Source: three-view drawing plus pictorial views. Frame: mm from the lowest corner of the part. A direction names the side the tool comes from. Give positions to 0.01 mm unless a question says otherwise; leave off trailing zeros. Loops run counter-clockwise (first coordinate to the right, second up) from the corner with the lowest first, then second, coordinate; pieces in that order, holes last.
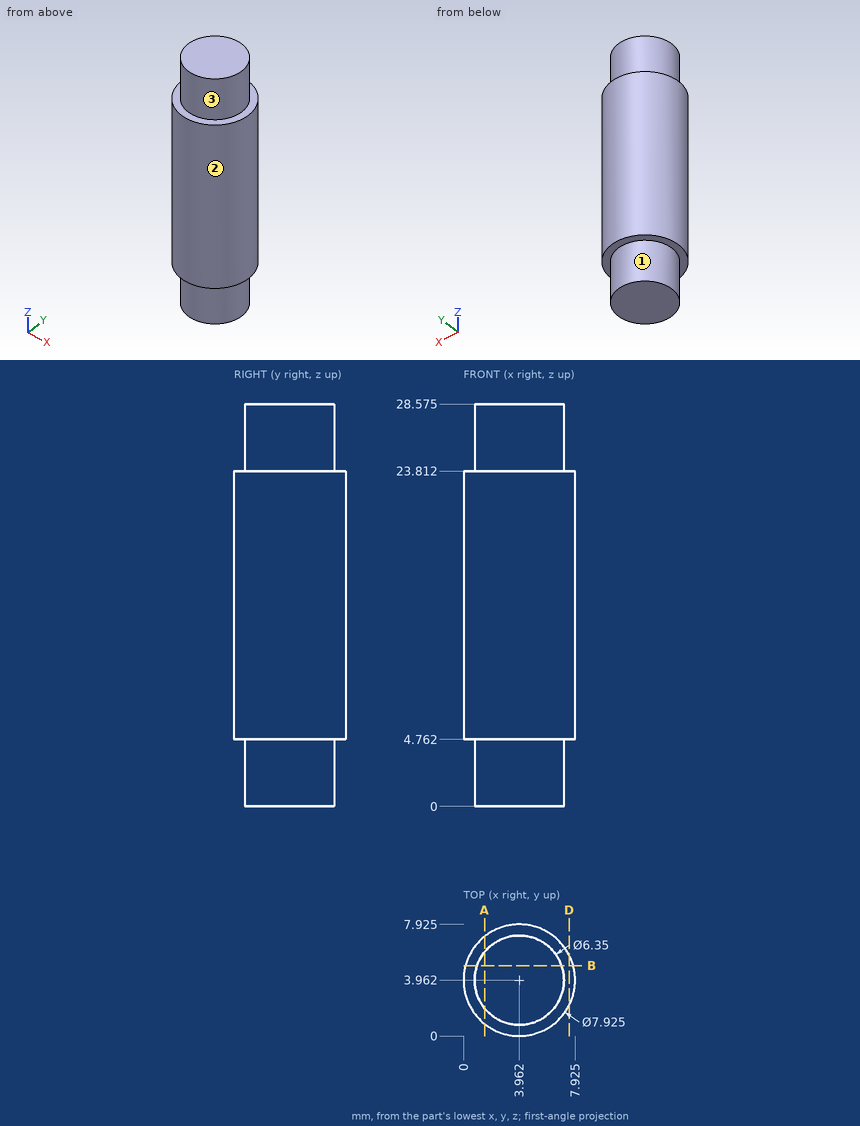
Q1. Reachability of the marked faces 1, 2 and 3 from +Z, -Z, +X, -X, +Y, -Y: full face, straight path, thin tool, end or side. Return the list, or none.
Q2. Section query A-A, the plane x = 1.5. Return loops of the section in (y, z) (1 decimal).
Q3. Material intervals for probe 1 along Y at (x, z) = (3.75, 23.75) (1 decimal); probe 2 along Z at (x, y) = (3.25, 0.75); probe 3 along X at (y, z) = (3.5, 1.5), sorted ascending.
Q4. Pin query (flat end, axial travel): pin 1 Ø1 at (x, z) = (3, 22) entering from -Y; pin 2 Ø4 at (y, z) = (1, 13) entering from +X; pin 3 Ø4 at (x, z) = (6.5, 3.5) entering from +Y. Return the tip coordinate at first contact, or that it passes through.
Q5. Section query B-B, the plane y = 5. Return loops of the section in (x, z) (1 decimal), and give its area (3 significant figures).
Q6. Section query D-D, the plane x = 7.5. Return loops of the section in (y, z).
Resolved:
1. face 1: -Z
1. face 2: +Z, -Z
1. face 3: +Z
2. outline: (0.9, 4.8) - (2, 4.8) - (2, 0) - (6, 0) - (6, 4.8) - (7.1, 4.8) - (7.1, 23.8) - (6, 23.8) - (6, 28.6) - (2, 28.6) - (2, 23.8) - (0.9, 23.8) - close
3. probe 1: y = 0 to 7.9
3. probe 2: z = 4.76 to 23.81
3. probe 3: x = 0.82 to 7.1
4. pin 1: stops at y = 0.03
4. pin 2: stops at x = 7.81
4. pin 3: stops at y = 7.8
5. outline: (0.1, 4.8) - (1, 4.8) - (1, 0) - (7, 0) - (7, 4.8) - (7.8, 4.8) - (7.8, 23.8) - (7, 23.8) - (7, 28.6) - (1, 28.6) - (1, 23.8) - (0.1, 23.8) - close
5. area: 203 mm2
6. outline: (2.18, 4.76) - (5.75, 4.76) - (5.75, 23.81) - (2.18, 23.81) - close
